Can you work these out from the model? Positions are in its coordinate system, mm. A direction names the side the tool comes from. Round coordinates to 2 decimals unless told otherwise and drop trailing zeros. Loops run counter-clockwise (first coordinate to the right, second up) from the corner with the lowest first, then second, coordinate; pieces in that order, holes last.
(1) Will these pins go through, and if not, where does the flat tip stop? pin 1 Ø1.5 at (y, z) = (31, 3) entering from -X; pin 2 Ø5 at (x, z) = (11.5, -3.5) entering from -Y; pin 3 Ø6 at (x, z) = (10, -1) entering from +Y.
(2) If I drill on line 1 along Y through (x, z) = (12.25, 0); line 2 along X through (y, z) = (26.25, -6); line 3 along Z through (x, y) = (13.5, 25.5), over which ranges is the centre line in solid material (lowest first)?
(3) I want a section at A-A on z = 0. Write out the boundary of the cut face in (x, y), plus the area to 3 significant figures.
(4) I want a section at C-C on x = 11.25. Write out the boundary of the cut face in (y, z), plus the area to 3 significant figures.
(5) I want a section at B-B on x = 14.75. Write out the boundary of the cut face in (y, z), plus the area to 3 significant figures.
(6) Which directions (+Z, -Z, +X, -X, +Y, -Y) give clear straight access to the entire face, cutting with the end or side of a thin tool? Please do faces 1 (the face through (6.5, 27, 2)), 2 (the face through (14.5, 23, 3)).
from build123d import *

# Parameters (mm, degrees)
CHAMFER1_SIZE = 0.5


with BuildPart() as part:
    # Sketch1 → Revolve1 (revolve)
    with BuildSketch(Plane.XY, mode=Mode.PRIVATE) as revolve1_sk:
        Polygon((6.5, 30.042572215), (14.5, 30.042572215), (14.5, 33.042572215), (17.5, 33.042572215), (17.5, 27.642572215), (6.5, 27.642572215), align=None)
    revolve(revolve1_sk.sketch.rotate(Axis((17.5, 26.042572215, 0), (-1, 0, 0)), 90), axis=Axis((17.5, 26.042572215, 0), (-1, 0, 0)))

    # Chamfer1
    chamfer1_edges = [part.edges().sort_by_distance(p)[0] for p in [
        (17.5, 26.042572215, 7),
        (14.5, 26.042572215, 7),
        (6.5, 26.042572215, 4),
        (17.5, 26.042572215, 1.6),
    ]]
    chamfer(chamfer1_edges, length=CHAMFER1_SIZE)


solid = part.part
Filled sheet:
1. pin 1: stops at x = 14.5
1. pin 2: stops at y = 22.17
1. pin 3: stops at y = 30.04
2. line 1: y = 22.04 to 24.44, 27.64 to 30.04
2. line 2: x = 14.5 to 17.5
2. line 3: z = -3.96 to -1.51, 1.51 to 3.96
3. outline: (6.5, 22.54) - (7, 22.04) - (14.5, 22.04) - (14.5, 19.54) - (15, 19.04) - (17, 19.04) - (17.5, 19.54) - (17.5, 23.94) - (17, 24.44) - (6.5, 24.44) - close; (6.5, 27.64) - (17, 27.64) - (17.5, 28.14) - (17.5, 32.54) - (17, 33.04) - (15, 33.04) - (14.5, 32.54) - (14.5, 30.04) - (7, 30.04) - (6.5, 29.54) - close
3. area: 69.8 mm2
4. outline: circle Ø8 at (26.04, 0); hole circle Ø3.2 at (26.04, 0)
4. area: 42.2 mm2
5. outline: circle Ø13.5 at (26.04, 0); hole circle Ø3.2 at (26.04, 0)
5. area: 135 mm2
6. face 1: +Z, -Z, -X, +Y, -Y
6. face 2: -X
